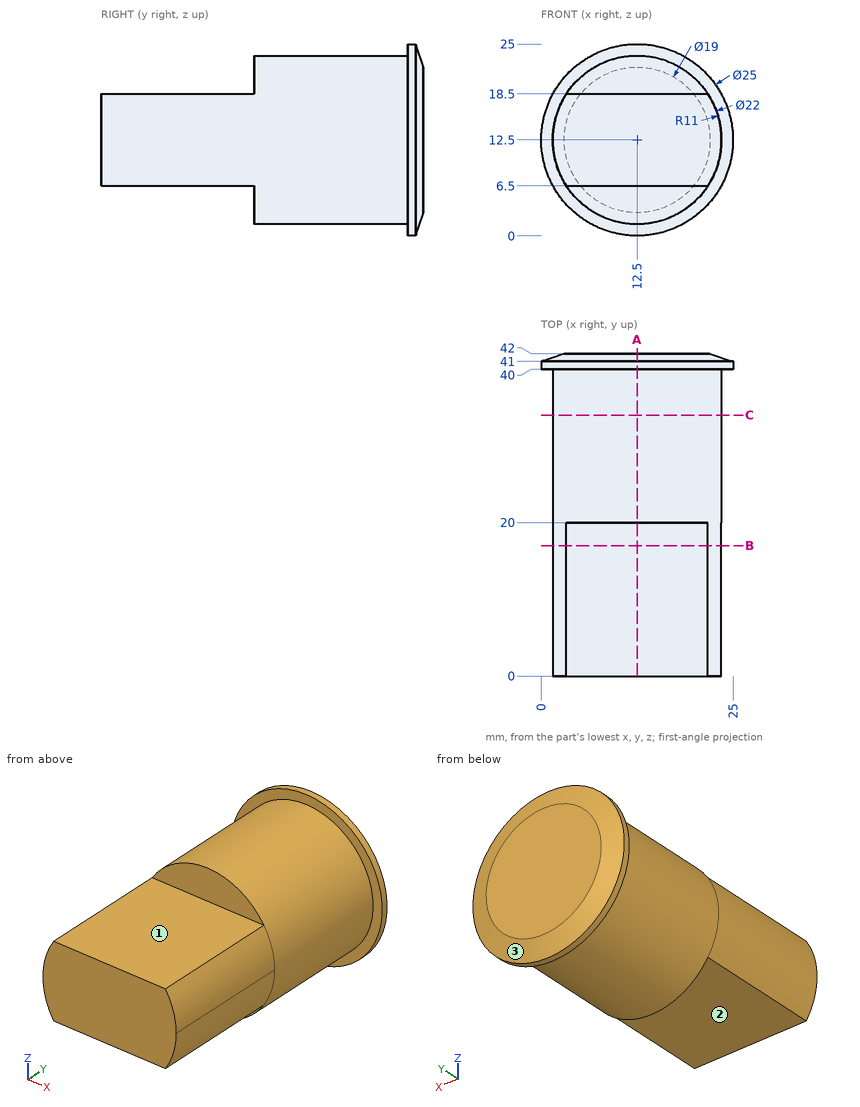
Here's the drawing with two shaded views (mm, measured from the low corner). I have some questions. A direction names the side the tool comes from. Coordinates: 2 decimals unless noted, no trailing zeros. Write each loop counter-clockwise with the first axis right and the second up, starting at its lowest first coordinate (ties: lowest second). Pieces come first, ordered by that corner, then holes. Notation, with made-up numbers: M 24,-22.5 L 67,-22.5 A11 cw 67,-18.5 Z; hole C -39,-36.5 d9. An arc over 180 degrees is marked long. Write item = value, one per line. Start each with the question number.
Q1. I'm going to push flat-ended pins straight in: pin 1 (5 mm diameter, centred on y = 33, z = 19, fed in from -X); pin 2 (2.5 mm diameter, centred on x = 15, z = 4, fed in from -Y); pin 3 (5 mm diameter, centred on x = 11.5, z = 10.5, fed in from -Y); pin 4 (5.5 mm diameter, centred on x = 10, y = 14, fed in from -Z). Where does each tip first touch, or does it pass through?
Q2. On a 3-axis mill with a long thin cutter (end or side, diameter ignored), from which of +Z, -Z, +X, -X, +Y, -Y can I reach the whole of each face in a straight line? I mean the marked faces 1, 2 and 3. Say none if no direction works.
Q3. If we section it at B-B, the plane y = 17: Write out the boundary of the cut face in (x, z), then the cut area to 3 significant figures.
Q4. If we section it at C-C, the plane y = 34: Write out the boundary of the cut face in (x, z).
Q5. If we section it at A-A, the plane x = 12.5: Write out the boundary of the cut face in (y, z).
Q6. If I drill on L1, parallel to Y at x = 9, z = 4; L2, parallel to Z at x = 20.25, y = 6.5; L3, parallel to Z at x = 12.75, y = 29.5, over which ranges is the centre line in solid material (lowest first)? Write a range as [from, to].
Check sheet entries:
q1.pin_1 = 2.25
q1.pin_2 = 20
q1.pin_3 = 0
q1.pin_4 = 6.5
q2.face_1 = +Z, +X, -X, -Y
q2.face_2 = -Z, +X, -X, -Y
q2.face_3 = +Y
q3.outline = M 3.28,6.5 L 21.72,6.5 A11 ccw 21.72,18.5 L 3.28,18.5 A11 ccw Z
q3.area = 250 mm²
q4.outline = C 12.5,12.5 d22
q5.outline = M 0,6.5 L 20,6.5 L 20,1.5 L 40,1.5 L 40,0 L 41,0 L 42,3 L 42,22 L 41,25 L 40,25 L 40,23.5 L 20,23.5 L 20,18.5 L 0,18.5 Z
q6.L1 = [20, 42]
q6.L2 = [6.5, 18.5]
q6.L3 = [1.5, 23.5]
